CAD build for the part. Positions are in the model's coordinates, mm. Face numbers are marked on the shaded views. A direction names the side the tool comes from. Give positions to 0.01 mm unless a question says otherwise; leave off trailing zeros. Loops run counter-clockwise (first coordinate to the right, second up) from the corner with the lowest first, then second, coordinate; pieces in that order, holes last. Notation, with made-up numbers: (87, 53) -> (139, 53) arc R16 ccw to (139, 83) -> close; hole circle Ø4 at (73, 82). An arc over 180 degrees is marked (long way). Use one line per item in the form item = value.
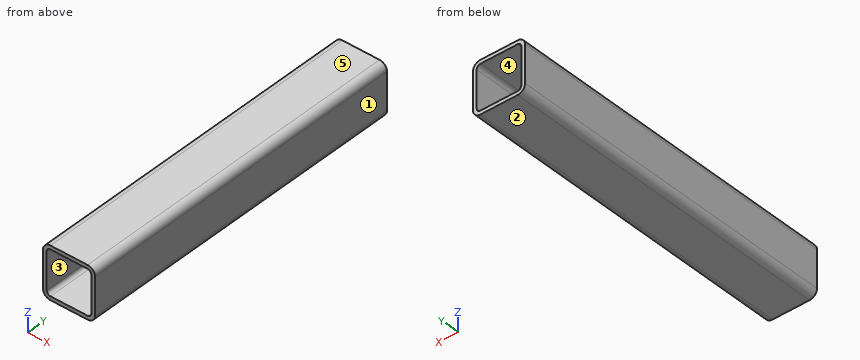
```python
from build123d import *

# Parameters (mm, degrees)
GB_T6728_2002_70_70_5_1_DEPTH = 455


with BuildPart() as part:
    # Sketch1 → 结构用冷弯空心方钢(gb t6728-2002) 70×70×5(1) (new body)
    with BuildSketch(Plane(origin=(0, 0, 0), x_dir=(-1, 0, 0), z_dir=(0, 1, 0))):
        with BuildLine():
            Line((-25, -35), (25, -35))
            ThreePointArc((25, -35), (32.071067812, -32.071067812), (35, -25))
            Line((35, -25), (35, 25))
            ThreePointArc((35, 25), (32.071067812, 32.071067812), (25, 35))
            Line((25, 35), (-25, 35))
            ThreePointArc((-25, 35), (-32.071067812, 32.071067812), (-35, 25))
            Line((-35, 25), (-35, -25))
            ThreePointArc((-35, -25), (-32.071067812, -32.071067812), (-25, -35))
        make_face()
        with BuildLine():
            Line((-25, -30), (25, -30))
            ThreePointArc((25, -30), (28.535533906, -28.535533906), (30, -25))
            Line((30, -25), (30, 25))
            ThreePointArc((30, 25), (28.535533906, 28.535533906), (25, 30))
            Line((25, 30), (-25, 30))
            ThreePointArc((-25, 30), (-28.535533906, 28.535533906), (-30, 25))
            Line((-30, 25), (-30, -25))
            ThreePointArc((-30, -25), (-28.535533906, -28.535533906), (-25, -30))
        make_face(mode=Mode.SUBTRACT)
    extrude(amount=GB_T6728_2002_70_70_5_1_DEPTH)


solid = part.part
```
1. Cut at A-A, the plane z = 12.5. Write the cut outline in (x, y).
Result sheet:
outline = (-35, 0) -> (-30, 0) -> (-30, 455) -> (-35, 455) -> close; (30, 0) -> (35, 0) -> (35, 455) -> (30, 455) -> close
2. Tool access for the marked faces 4 and 5: list every direction of +Z, -Z, +X, -X, +Y, -Y with a clear straight run to the whole face (end or side of a thin tool).
Result sheet:
face_4 = +Y, -Y
face_5 = +Z, +X, -X, +Y, -Y
3. Drill centre lines: line 1 (X direction, y = 178, z = -13.5); line 2 (X direction, y = 360, z = -28). Where is each one in solid material? Low to high.
Result sheet:
line_1 = -35 to -30, 30 to 35
line_2 = -34.54 to -29, 29 to 34.54
4. Mould opens along Z. For the marked faces 1, 2 and 3 say: pulls with the +Z half, pulls with the -Z half, needs draft (parallel to the pull), parting line crosses it, or undercut.
Result sheet:
face_1 = needs draft
face_2 = pulls with the -Z half
face_3 = undercut
5. Cut at B-B, the plane x = -13. Write the cut outline in (y, z).
Result sheet:
outline = (0, -35) -> (455, -35) -> (455, -30) -> (0, -30) -> close; (0, 30) -> (455, 30) -> (455, 35) -> (0, 35) -> close
6. Cut at C-C, the plane y = 57. Write the cut outline in (x, z), then the cut area to 3 significant figures.
Result sheet:
outline = (-35, -25) arc R10 ccw to (-25, -35) -> (25, -35) arc R10 ccw to (35, -25) -> (35, 25) arc R10 ccw to (25, 35) -> (-25, 35) arc R10 ccw to (-35, 25) -> close; hole (-30, -25) arc R5 ccw to (-25, -30) -> (25, -30) arc R5 ccw to (30, -25) -> (30, 25) arc R5 ccw to (25, 30) -> (-25, 30) arc R5 ccw to (-30, 25) -> close
area = 1,240 mm^2
